The listing builds one solid part. Answer for the finished solid, in the listing's coordinates (mm). Coordinates: 2 decimals unless noted, no trailing zeros. Order: outer loops, then holes, each group sorted by start corner. A loop starts at its lowest first (then second) coordinate and runs counter-clockwise, first axis right, second up. Notation, with made-up numbers: (28.25, 46) -> (86.25, 46) arc R14 cw to (86.25, 68) -> close; hole circle Ø1 at (84.25, -39). An arc over 180 degrees is marked (long way). Return JSON: item names as keys, results as strings.
from build123d import *

# Parameters (mm, degrees)
SKETCH_1_R             = 12.5
EXTRUDE_1_DEPTH        = 605
HOLE_WIZARD_M8_1_D     = 6.8
HOLE_WIZARD_M8_1_DEPTH = 22.25
HOLE_WIZARD_M8_1_TIP   = 2.042926105
CHAMFER_1_SIZE         = 0.5
HOLE_WIZARD_M8_2_D     = 6.8
HOLE_WIZARD_M8_2_DEPTH = 19.75
HOLE_WIZARD_M8_2_TIP   = 2.042926105


with BuildPart() as part:
    # 草图1 → 凸台-拉伸1 (new body)
    with BuildSketch(Plane.XY):
        Circle(SKETCH_1_R)
    extrude(amount=EXTRUDE_1_DEPTH)

    # M8 螺纹孔1
    with Locations(Plane(origin=(0, 0, 0), x_dir=(1, 0, 0), z_dir=(0, 0, -1))):
        with Locations((0, 0)):
            Hole(HOLE_WIZARD_M8_1_D / 2, depth=HOLE_WIZARD_M8_1_DEPTH)
            with Locations((0, 0, -(HOLE_WIZARD_M8_1_DEPTH + HOLE_WIZARD_M8_1_TIP / 2))):  # 118° drill point
                Cone(0, HOLE_WIZARD_M8_1_D / 2, HOLE_WIZARD_M8_1_TIP, mode=Mode.SUBTRACT)

    # 倒角1
    chamfer_1_edges = [part.edges().sort_by_distance(p)[0] for p in [
        (-12.5, 0, 0),
        (-12.5, 0, 605),
    ]]
    chamfer(chamfer_1_edges, length=CHAMFER_1_SIZE)

    # M8 螺纹孔2
    with Locations(Plane.XY.offset(605)):
        with Locations((0, 0)):
            Hole(HOLE_WIZARD_M8_2_D / 2, depth=HOLE_WIZARD_M8_2_DEPTH)
            with Locations((0, 0, -(HOLE_WIZARD_M8_2_DEPTH + HOLE_WIZARD_M8_2_TIP / 2))):  # 118° drill point
                Cone(0, HOLE_WIZARD_M8_2_D / 2, HOLE_WIZARD_M8_2_TIP, mode=Mode.SUBTRACT)


solid = part.part
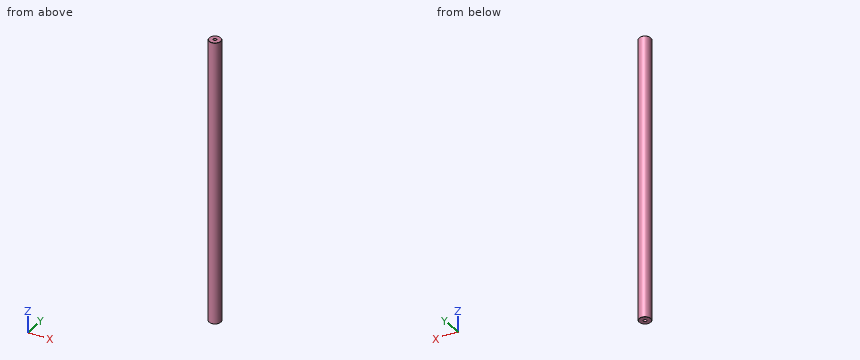
1. Each of these flat-tipped pins is pushed along its axis until it touches: pin 1 Ø8 at (x, z) = (9.5, 185.5) entering from -Y (3 decimals); pin 2 Ø11 at (x, y) = (0, 0) entering from -Z; pin 3 Ø1 at (y, z) = (6, 106) entering from +X (3 decimals); pin 4 Ø6 at (y, z) = (-4.5, 497) entering from +X. Where does it stop, or does it pass through?
Answer block:
{"pin 1": "stops at y = -11.225", "pin 2": "stops at z = 0", "pin 3": "stops at x = 11.225", "pin 4": "stops at x = 12.41"}
2. Consider line 1 (Y direction, x = 0, z = 7.25); line 2 (Y direction, x = 0, z = 365); line 3 (X direction, y = 1, z = 264.5). Determine where each line is inside the solid, lowest interval first. Write a range as from..to.
Answer block:
{"line 1": "y = -12.5..-3.4, 3.4..12.5", "line 2": "y = -12.5..12.5", "line 3": "x = -12.46..12.46"}
3. The part is cut by section A-A on z = 146. Give the vertices of the cut face in (x, y), and give its area (3 significant figures).
Answer block:
{"outline": "circle Ø25 at (0, 0)", "area": "491 mm2"}
